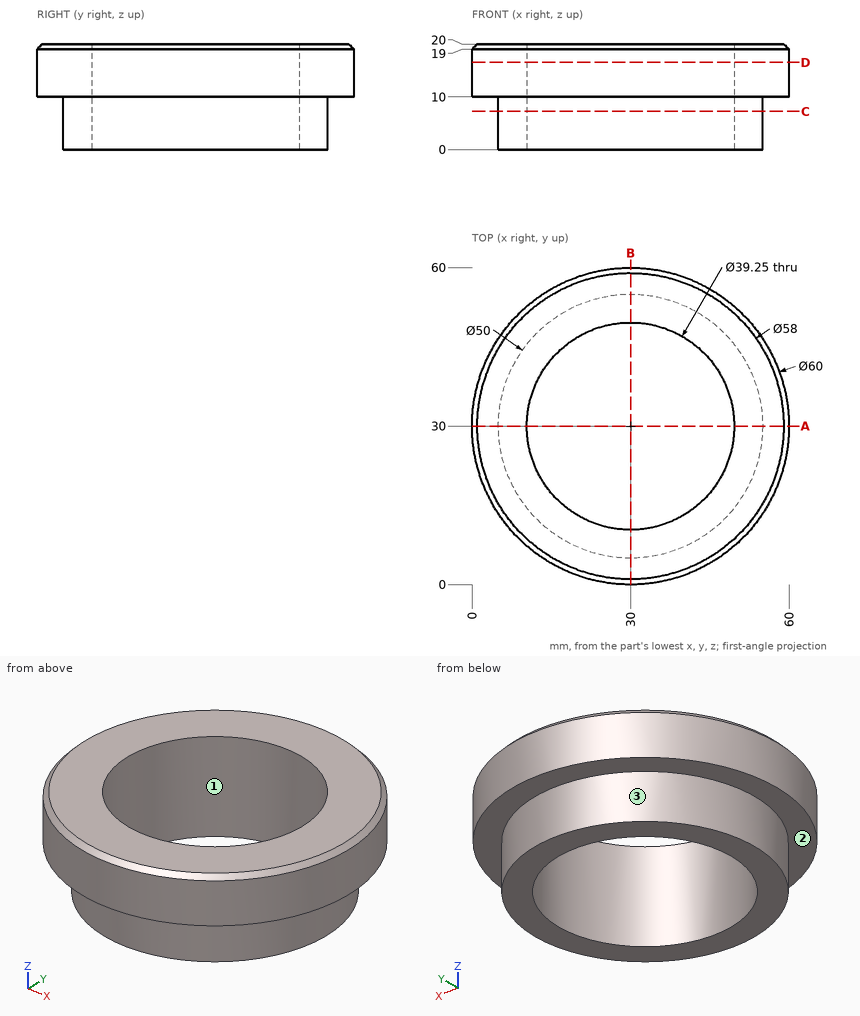
For this review, use the dimensioned drawing (mm, ordinates from the lowest corner) and the shaded views. Coordinates: 2 decimals unless noted, no trailing zeros. Loops run counter-clockwise (first coordinate to the right, second up) from the corner with the lowest first, then second, coordinate; pieces in that order, holes last. Notation, with made-up numbers: (44, -39) - (52, -39) arc R32 cw to (52, -9) - close; hole circle Ø2 at (20.25, 4). An arc over 180 degrees is marked (long way). Use CSV: the item, a comma, the result in double quotes. Start each with the question number.
1) The part is to be moulded in two halves that separate along X. For the marked faces 1, 2 and 3, say which applies: +X half, -X half, draft (parallel to the pull), parting line (faces both ways), or undercut.
2) Consider section D-D on z = 16.5. Write out the cut boundary in (x, y) (3 decimals).
3) Wall thickness on L1, parallel to Y at x = 30, z = 10.5 (3 decimals); L2, parallel to Y at x = 30, z = 4.25 (3 decimals); L3, parallel to X at y = 25.5, z = 12: over which ranges is each line inside the solid? List them lowest first. Write a range as from..to.
4) Consider section A-A on y = 30. Write out the cut boundary in (x, z) (3 decimals).
5) Consider section C-C on z = 7.25. Write out the cut boundary in (x, y) (3 decimals).
6) For pin 1 Ø1.5 at (y, z) = (9.5, 6) entering from -X; pin 2 Ø6 at (x, z) = (52, 10) entering from +Y; pin 3 Ø8 at (x, z) = (49.5, 7) entering from +Y; pin 4 Ø8 at (x, y) = (8.5, 21) entering from -Z, all flat-tipped, find the tip position at first contact; note any pin that passes through.
Geometry says:
1,face 1,"undercut"
1,face 2,"draft"
1,face 3,"parting line"
2,outline,"circle Ø60 at (30, 30); hole circle Ø39.25 at (30, 30)"
3,L1,"0..10.375, 49.625..60"
3,L2,"5..10.375, 49.625..55"
3,L3,"0.34..10.9, 49.1..59.66"
4,outline,"(0, 10) - (5, 10) - (5, 0) - (10.375, 0) - (10.375, 20) - (1, 20) - (0, 19) - close; (49.625, 0) - (55, 0) - (55, 10) - (60, 10) - (60, 19) - (59, 20) - (49.625, 20) - close"
5,outline,"circle Ø50 at (30, 30); hole circle Ø39.25 at (30, 30)"
6,pin 1,"x = 14.67"
6,pin 2,"y = 53.22"
6,pin 3,"y = 54.82"
6,pin 4,"z = 0"
